from build123d import *

# Parameters (mm, degrees)
SKETCH1_R           = 9.25
SKETCH1_R_2         = 3.5
BOSS_EXTRUDE1_DEPTH = 1.5


with BuildPart() as part:
    # Sketch1 → Boss-Extrude1 (new, symmetric)
    with BuildSketch(Plane.XY):
        Polygon((-20, 117), (-17, 120), (17, 120), (20, 117), (20, -117), (17, -120), (-17, -120), (-20, -117), align=None)
        with Locations((0, 100)):
            Circle(SKETCH1_R, mode=Mode.SUBTRACT)
        with Locations((0, -105)):
            Circle(SKETCH1_R_2, mode=Mode.SUBTRACT)
        with Locations((0, -85)):
            Circle(SKETCH1_R_2, mode=Mode.SUBTRACT)
        with Locations((0, -65)):
            Circle(SKETCH1_R_2, mode=Mode.SUBTRACT)
        with Locations((0, -45)):
            Circle(SKETCH1_R_2, mode=Mode.SUBTRACT)
        with Locations((0, -25)):
            Circle(SKETCH1_R_2, mode=Mode.SUBTRACT)
        with Locations((0, -5)):
            Circle(SKETCH1_R_2, mode=Mode.SUBTRACT)
    extrude(amount=BOSS_EXTRUDE1_DEPTH, both=True)


solid = part.part
Geometry: final body of the model. Coordinates: model frame, mm. Give positions to 0.01 mm unless a question says otherwise; leave off trailing zeros. Write each loop counter-clockwise with the first axis right and the second up, starting at its lowest first coordinate (ties: lowest second). Pieces come first, ordered by that corner, then holes. Notation, with made-up numbers: (68, 25) - (80, 25) arc R16 cw to (80, 56) - close; hole circle Ø11 at (73.5, -25). An arc over 180 degrees is marked (long way). Return JSON: item names as keys, results as strings. Group by question number.
1) Line query: line 1 (Y direction, x = -8, z = -0.35); line 2 (X direction, y = 107, z = 1.3); line 3 (Y direction, x = 5, z = 0.25). Output: solid intervals per line, ascending.
2) Section D-D on y = -5. Return the cut outline in (x, z), plus the area to 3 significant figures.
3) Mould query, pull axis Y, two halves, no side actions, for faces 1 (the flat face through (0, 2, 1.5)), 2 (the cylindrical face through (-2.58, -62.635, -0.021)). Classes: released by +Y, released by -Y, zero draft, split by the parting line, or undercut.
4) Section C-C on z = 0.15. Return the cut outline in (x, y), plus the area to 3 significant figures.
5) Section A-A on y = 100. Return the cut outline in (x, z), plus the area to 3 significant figures.
6) Section B-B on x = 0. State how many separate pieces and enclosed holes the cut face has, plus the area to 4 significant figures.
Filled in:
{
 "1": {"line 1": "y = -120 to 95.36, 104.64 to 120", "line 2": "x = -20 to -6.05, 6.05 to 20", "line 3": "y = -120 to 92.22, 107.78 to 120"},
 "2": {"outline": "(-20, -1.5) - (-3.5, -1.5) - (-3.5, 1.5) - (-20, 1.5) - close; (3.5, -1.5) - (20, -1.5) - (20, 1.5) - (3.5, 1.5) - close", "area": "99.0 mm^2"},
 "3": {"face 1": "zero draft", "face 2": "undercut"},
 "4": {"outline": "(-20, -117) - (-17, -120) - (17, -120) - (20, -117) - (20, 117) - (17, 120) - (-17, 120) - (-20, 117) - close; hole circle Ø18.5 at (0, 100); hole circle Ø7 at (0, -105); hole circle Ø7 at (0, -85); hole circle Ø7 at (0, -65); hole circle Ø7 at (0, -45); hole circle Ø7 at (0, -25); hole circle Ø7 at (0, -5)", "area": "9,080 mm^2"},
 "5": {"outline": "(-20, -1.5) - (-9.25, -1.5) - (-9.25, 1.5) - (-20, 1.5) - close; (9.25, -1.5) - (20, -1.5) - (20, 1.5) - (9.25, 1.5) - close", "area": "64.5 mm^2"},
 "6": {"separate pieces": "8", "enclosed holes": "0", "area": "538.5 mm^2"}
}
